Drawing for the job (mm, zero at the part's lowest x, y, z). Coordinates: 2 decimals unless noted, no trailing zeros. Loops run counter-clockwise (first coordinate to the right, second up) from the corner with the lowest first, then second, coordinate; pieces in that order, holes last. Notation, with made-up numbers: (87.5, 47.25) - (107.5, 47.25) arc R14 cw to (107.5, 65.25) - close; hole circle Ø4 at (50, 27.5). An arc over 180 degrees is marked (long way). Put each result on its own line as item: value.
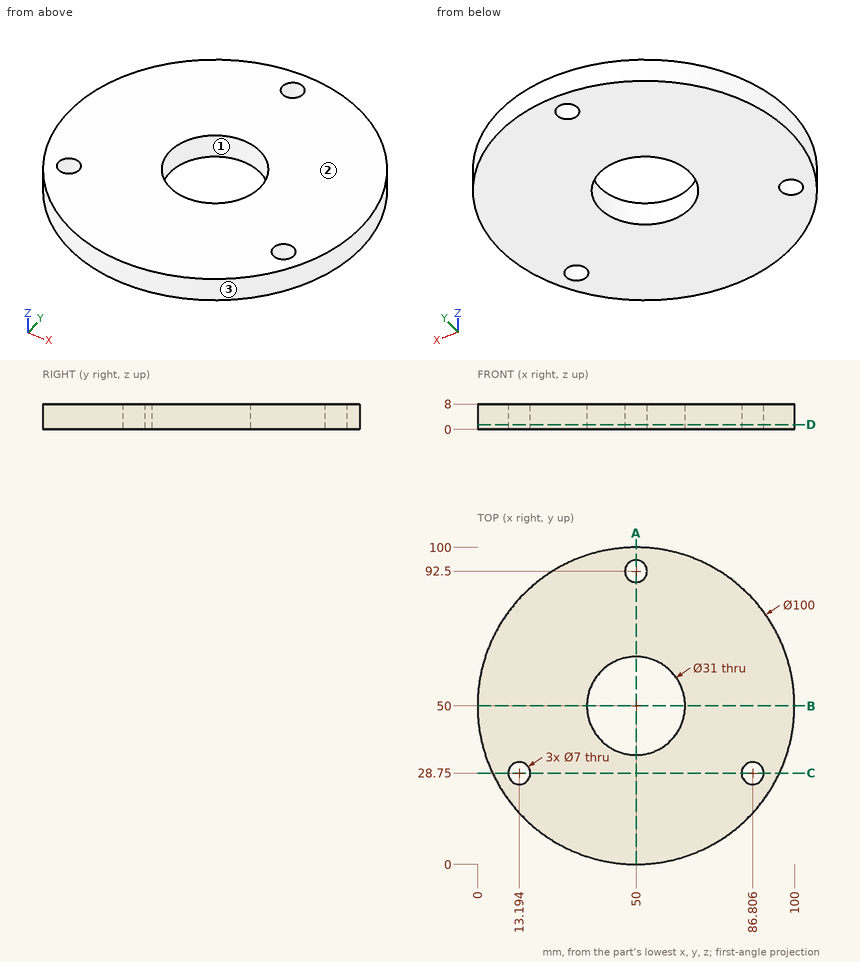
Q1. Slice it at B-B, the plane y = 50. Give the cut face in (x, z), then the cut area to 3 significant figures.
Determined:
outline: (0, 0) - (34.5, 0) - (34.5, 8) - (0, 8) - close; (65.5, 0) - (100, 0) - (100, 8) - (65.5, 8) - close
area: 552 mm2
Q2. Mould opens along X. For the marked faces 1, 2 and 3 say: +X half, -X half, draft (parallel to the pull), parting line (faces both ways), or undercut.
Determined:
face 1: undercut
face 2: draft
face 3: parting line
Q3. Slice it at A-A, the plane x = 50. Give the cut face in (y, z).
Determined:
outline: (0, 0) - (34.5, 0) - (34.5, 8) - (0, 8) - close; (65.5, 0) - (89, 0) - (89, 8) - (65.5, 8) - close; (96, 0) - (100, 0) - (100, 8) - (96, 8) - close
Q4. Pin check, flat tips, straight feed: pin 1 Ø5.5 at (x, y) = (50, 92.5) entering from +Z; pin 2 Ø1 at (y, z) = (78.5, 2) entering from -X; pin 3 Ø11 at (x, y) = (86.81, 28.75) entering from +Z; pin 4 Ø2 at (x, z) = (89.5, 6) entering from -Y. Stop position of each tip, or through.
Determined:
pin 1: through
pin 2: x = 8.58
pin 3: z = 8
pin 4: y = 18.1
Q5. Slice it at C-C, the plane y = 28.75. Give the cut face in (x, z), then the cut area to 3 significant figures.
Determined:
outline: (4.74, 0) - (9.69, 0) - (9.69, 8) - (4.74, 8) - close; (16.69, 0) - (83.31, 0) - (83.31, 8) - (16.69, 8) - close; (90.31, 0) - (95.26, 0) - (95.26, 8) - (90.31, 8) - close
area: 612 mm2
Q6. Wall check: L1, parallel to Y at x = 50, z = 2; L2, parallel to X at y = 50.5, z = 4.25; L3, parallel to X at y = 26.5, z = 6.5 (1 decimal). Give the ranges that are in metal, low to high. Write a range as from..to.
Determined:
L1: 0..34.5, 65.5..89, 96..100
L2: 0..34.51, 65.49..100
L3: 5.9..10.5, 15.9..84.1, 89.5..94.1
Q7. Slice it at D-D, the plane z = 1.5. Give the cut face in (x, y).
Determined:
outline: circle Ø100 at (50, 50); hole circle Ø7 at (13.19, 28.75); hole circle Ø31 at (50, 50); hole circle Ø7 at (50, 92.5); hole circle Ø7 at (86.81, 28.75)
